Read the model definition and answer for the solid it produces. Units are mm, in the model's axes. Face numbers are marked on the shaded views. Give positions to 0.01 mm unless a question says otherwise; leave off trailing zeros. Loops run counter-clockwise (first coordinate to the right, second up) from the corner with the lowest first, then second, coordinate; pieces in that order, holes last.
(1) Each of these flat-tipped pins is pushed along its axis until it touches: P1, Ø6, axis at x = -4, z = 7.5, coming from the +Y side; P2, Ø4, axis at x = 3, z = 8, coming from the -Y side. Where does it stop, or does it pass through?
(2) Find section A-A, the plane x = 0. Write down the section's boundary in (y, z).
(3) Straight lines are drawn through the part: probe 1 along Y at (x, z) = (0, 9.5); probe 2 along X at (y, z) = (114.5, 11); probe 3 along Y at (x, z) = (2, 4.75). For each, find the intervals that lie inside material, in ascending order.
(4) Determine the mould class of the marked faces 1, 2, 3 and 4 for opening direction X: pulls with the +X half, pulls with the -X half, needs draft (parallel to the pull), parting line crosses it, or undercut.
(5) Find section C-C, the plane y = 113. Write down the section's boundary in (x, z).
(6) Find section B-B, the plane z = 13. Write down the section's boundary in (x, y), then the cut area to 3 significant figures.
```python
from build123d import *

# Parameters (mm, degrees)
EXTRUDE_1_DEPTH     = 15
SKETCH_2_R          = 7
SKETCH_2_R_2        = 10
CUT_EXTRUDE_1_DEPTH = 132.719398723


with BuildPart() as part:
    # 草图1 → 凸台-拉伸1 (new body)
    with BuildSketch(Plane.XY):
        with BuildLine():
            Line((-15, 0), (-15, 115))
            ThreePointArc((-15, 115), (0, 130), (15, 115))
            Line((15, 115), (15, 0))
            ThreePointArc((15, 0), (0, -15), (-15, 0))
        make_face()
    extrude(amount=EXTRUDE_1_DEPTH)

    # 草图2 → 切除-拉伸1 (cut, through all)
    with BuildSketch(Plane.XY.offset(15)):
        with Locations((0, 115)):
            Circle(SKETCH_2_R)
        Circle(SKETCH_2_R_2)
    extrude(amount=-CUT_EXTRUDE_1_DEPTH, mode=Mode.SUBTRACT)


solid = part.part
```
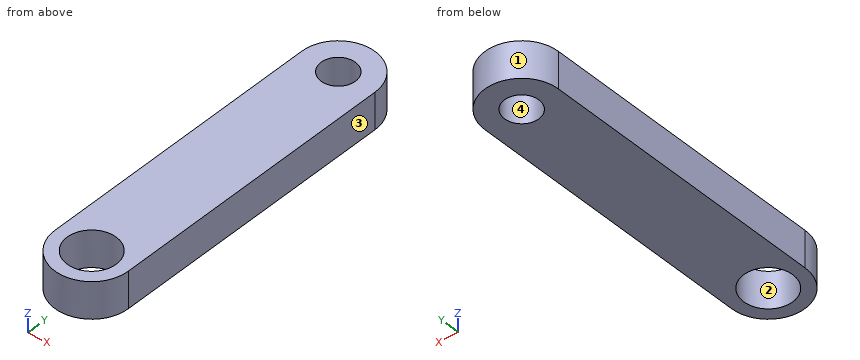
Entries:
1. P1: stops at y = 129.97
1. P2: stops at y = -14.97
2. outline: (-15, 0) - (-10, 0) - (-10, 15) - (-15, 15) - close; (10, 0) - (108, 0) - (108, 15) - (10, 15) - close; (122, 0) - (130, 0) - (130, 15) - (122, 15) - close
3. probe 1: y = -15 to -10, 10 to 108, 122 to 130
3. probe 2: x = -15 to -6.98, 6.98 to 15
3. probe 3: y = -14.87 to -9.8, 9.8 to 108.29, 121.71 to 129.87
4. face 1: parting line crosses it
4. face 2: undercut
4. face 3: pulls with the +X half
4. face 4: undercut
5. outline: (-15, 0) - (-6.71, 0) - (-6.71, 15) - (-15, 15) - close; (6.71, 0) - (15, 0) - (15, 15) - (6.71, 15) - close
6. outline: (-15, 0) arc R15 ccw to (15, 0) - (15, 115) arc R15 ccw to (-15, 115) - close; hole circle Ø20 at (0, 0); hole circle Ø14 at (0, 115)
6. area: 3,690 mm2
